Could you check a few things on this model? Use its own coordinates, in mm. Round coordinates to 2 decimals unless told otherwise and drop trailing zeros. Write each loop counter-clockwise with the first axis right and the second up, starting at its lowest first coordinate (ties: lowest second). Pieces come first, ordered by that corner, then holes. Notation, with made-up numbers: (81.5, -23) -> (96.5, -23) arc R11 cw to (96.5, -10) -> close; hole circle Ø1 at (-7, 81). An arc over 180 degrees is marked (long way). Return JSON: item names as keys, results as strings.
from build123d import *

# Parameters (mm, degrees)
SKETCH_1_W                  = 65
SKETCH_1_H                  = 10
EXTRUDE_1_DEPTH             = 116.5
HOLE_WIZARD_M4_1_AT_2_COUNT = 2
HOLE_WIZARD_M4_1_AT_2_PITCH = 50
HOLE_WIZARD_M4_1_2_D        = 4.5


with BuildPart() as part:
    # 草图1 → 凸台-拉伸1 (new, symmetric)
    with BuildSketch(Plane(origin=(0, 0, 0), x_dir=(1, 0, 0), z_dir=(0, 1, 0))):
        Rectangle(SKETCH_1_W, SKETCH_1_H)
    extrude(amount=EXTRUDE_1_DEPTH, both=True)

    # 草图3 → Hole Wizard M4 _1 (revolve, cut)
    with BuildSketch(Plane(origin=(25, 116.5, 0), x_dir=(0, 0, 1), z_dir=(1, 0, 0))):
        Polygon((0, 0), (0, 11.091420021), (1.65, 10.1), (1.65, 0), align=None)
    hole_wizard_m4_1 = revolve(axis=Axis((25, 122.85, 0), (0, -1, 0)), mode=Mode.SUBTRACT)

    # Hole Wizard M4 _1 at 2: Hole Wizard M4 _1 ×2
    with Locations(*[(-i * HOLE_WIZARD_M4_1_AT_2_PITCH, 0, 0) for i in range(1, HOLE_WIZARD_M4_1_AT_2_COUNT)]):
        add(hole_wizard_m4_1, mode=Mode.SUBTRACT)

    # 镜向1: Hole Wizard M4 _1 across plane
    add(hole_wizard_m4_1.mirror(Plane.ZX), mode=Mode.SUBTRACT)

    # 镜向1 copy 1 sketch → 镜向1 copy 1 (revolve, cut)
    with BuildSketch(Plane(origin=(-25, -116.5, 0), x_dir=(0, 0, 1), z_dir=(1, 0, 0))):
        Polygon((0, 0), (0, -11.091420021), (1.65, -10.1), (1.65, 0), align=None)
    revolve(axis=Axis((-25, -122.85, 0), (0, -1, 0)), mode=Mode.SUBTRACT)

    # Hole Wizard M4 _1 2 (through all)
    with Locations(Plane(origin=(0, 0, -5), x_dir=(-1, 0, 0), z_dir=(0, 0, -1))):
        with Locations((25, 21.5), (-25, 21.5)):
            Hole(HOLE_WIZARD_M4_1_2_D / 2)


solid = part.part
1) If I drill on probe 1 along X at (y, z) = (114, 0); probe 2 along Z at (x, y) = (25, 109); probe 3 along Y at (x, z) = (25, 2.25), over which ranges is the centre line in solid material (lowest first)? Write a range as [from, to].
Return value:
{"probe 1": "[-32.5, -26.65], [-23.35, 23.35], [26.65, 32.5]", "probe 2": "[-5, -1.65], [1.65, 5]", "probe 3": "[-116.5, 19.25], [23.75, 116.5]"}
2) Thinking about a two-plate mould opening in X: for faces 1 (the face through (-32.5, 2, 0)), 2 (the face through (-23.962, 19.504, 0.07)), 3 (the face through (0, 2, 5)), which applies, pulls with the +X half, pulls with the -X half, needs draft (parallel to the pull), parting line crosses it, or undercut?
Return value:
{"face 1": "pulls with the -X half", "face 2": "undercut", "face 3": "needs draft"}
3) I want a section at A-A, the plane y = 21.5. Please give me the cut outline in (x, z), and give its area (3 significant figures).
Return value:
{"outline": "(-32.5, -5) -> (-27.25, -5) -> (-27.25, 5) -> (-32.5, 5) -> close; (-22.75, -5) -> (22.75, -5) -> (22.75, 5) -> (-22.75, 5) -> close; (27.25, -5) -> (32.5, -5) -> (32.5, 5) -> (27.25, 5) -> close", "area": "560 mm²"}
4) Will these pins go through, and if not, where does the flat tip stop? pin 1 Ø6 at (x, y) = (25, 21.5) entering from -Z; pin 2 Ø2 at (x, z) = (25, 0) entering from -Y; pin 3 Ø3 at (x, z) = (-25, 0) entering from -Y.
Return value:
{"pin 1": "z = -5", "pin 2": "y = -106.01", "pin 3": "y = -106.31"}
